Read the model definition and answer for the solid it produces. Units are mm, in the model's axes. A direction names the side the tool comes from. Coordinates: 2 decimals unless noted, no trailing zeros. Write each loop counter-clockwise with the first axis right and the second up, starting at its lowest first coordinate (ties: lowest second). Pieces come first, ordered by that corner, then holes.
Item 1: Straight lines are drawn through the part: probe 1 along Z at (x, y) = (163, 14.5); probe 2 along X at (y, z) = (22, 67); probe 3 along X at (y, z) = (21, 66.5). For each, find the intervals that lie inside material, in ascending order.
Item 2: Section B-B (z = 62.5) is taken. Give the vertices of the cut face in (x, y).
Item 3: Determine the mould class of faces 4 (the face through (151.284, 25, 35)), 5 (the face through (59.284, 24, 5)), 6 (the face through (168.441, 22.825, 5.07)) for opening direction X: released by +X, released by -X, zero draft, split by the parting line, or undercut.
Item 4: A tool of negligible diameter and unlimited length cuts with its end or side. For faces 1 (the face through (185.28, 24.75, 65.07)), 2 (the face through (169, 25, 10)), 3 (the face through (86.382, 24.269, 59.145)), from which of +Z, -Z, +X, -X, +Y, -Y can it reach the whole face along a straight path? Write none if from no direction.
Item 5: Section A-A (y = 35) is taken. Give the vertices of the cut face in (x, z).
Item 6: Each of these flat-tipped pins is pushed along its axis until it touches: P1, Ø11, axis at y = 22, z = 5.5, coming from the -X side; P2, Ø12, axis at y = 23, z = 38, coming from the +X side; P3, Ø3, axis at y = 26.5, z = 7.5, coming from the +X side. Where does it stop, or does it pass through?
Item 7: Section C-C (z = 27.5) is taken. Give the vertices of the cut face in (x, y).
from build123d import *

# Parameters (mm, degrees)
SKETCH_1_W             = 120
SKETCH_1_H             = 40
EXTRUDE_1_DEPTH        = 70
SKETCH_2_R             = 3
CUT_EXTRUDE_1_DEPTH    = 198.553816398
SKETCH_3_W             = 47.323469883
SKETCH_3_H             = 50
CUT_EXTRUDE_2_DEPTH    = 197.577989194
FILLET_1_R             = 3
SKETCH_4_W             = 12
SKETCH_4_H             = 40
EXTRUDE_2_DEPTH        = 10
SKETCH_5_W             = 12
SKETCH_5_H             = 40
EXTRUDE_3_DEPTH        = 10
SKETCH_6_R             = 3
EXTRUDE_4_DEPTH        = 10
SKETCH_7_R             = 4.5
CUT_EXTRUDE_3_DEPTH    = 10
CHAMFER_1_SIZE         = 2
HOLE_WIZARD_M8_1_D     = 9
HOLE_WIZARD_M8_1_DEPTH = 19.75
HOLE_WIZARD_M8_1_TIP   = 2.703872786


with BuildPart() as part:
    # 草图1 → 凸台-拉伸1 (new body)
    with BuildSketch(Plane.XY):
        with Locations((119.284427197, 24.548900527)):
            Rectangle(SKETCH_1_W, SKETCH_1_H)
    extrude(amount=EXTRUDE_1_DEPTH)

    # 草图2 → 切除-拉伸1 (cut, through all)
    with BuildSketch(Plane.XY.offset(70)):
        with Locations((74.284427197, 24.548900527)):
            Circle(SKETCH_2_R)
        with Locations((164.284427197, 24.548900527)):
            Circle(SKETCH_2_R)
    extrude(amount=-CUT_EXTRUDE_1_DEPTH, mode=Mode.SUBTRACT)

    # 草图3 → 切除-拉伸2 (cut, through all)
    with BuildSketch(Plane(origin=(0, 44.548900527, 0), x_dir=(1, 0, 0), z_dir=(0, 1, 0))):
        with Locations((174.946162139, -35)):
            Rectangle(SKETCH_3_W, SKETCH_3_H)
        with Locations((63.622692255, -35)):
            Rectangle(SKETCH_3_W, SKETCH_3_H)
    extrude(amount=-CUT_EXTRUDE_2_DEPTH, mode=Mode.SUBTRACT)

    # 圆角1
    fillet_1_edges = [part.edges().sort_by_distance(p)[0] for p in [
        (151.284427197, 24.548900527, 10),
        (151.284427197, 24.548900527, 60),
        (87.284427197, 24.548900527, 60),
        (87.284427197, 24.548900527, 10),
    ]]
    fillet(fillet_1_edges, radius=FILLET_1_R)

    # 草图4 → 凸台-拉伸2 (add)
    with BuildSketch(Plane(origin=(0, 0, 60), x_dir=(-1, 0, 0), z_dir=(0, 0, -1))):
        with Locations((-185.284427197, 24.548900527)):
            Rectangle(SKETCH_4_W, SKETCH_4_H)
    extrude(amount=-EXTRUDE_2_DEPTH)

    # 草图5 → 凸台-拉伸3 (add)
    with BuildSketch(Plane.XY.offset(70)):
        with Locations((53.284427197, 24.548900527)):
            Rectangle(SKETCH_5_W, SKETCH_5_H)
    extrude(amount=-EXTRUDE_3_DEPTH)

    # 草图6 → 凸台-拉伸4 (add)
    with BuildSketch(Plane.XY.offset(70)):
        with Locations((74.284427197, 24.548900527)):
            Circle(SKETCH_6_R)
        with Locations((164.284427197, 24.548900527)):
            Circle(SKETCH_6_R)
    extrude(amount=-EXTRUDE_4_DEPTH)

    # 草图7 → 切除-拉伸3 (cut)
    with BuildSketch(Plane.XY.offset(70)):
        with Locations((57.784427197, 24.548900527)):
            Circle(SKETCH_7_R)
    cut_extrude_3 = extrude(amount=-CUT_EXTRUDE_3_DEPTH, mode=Mode.SUBTRACT)

    # 镜向2: 切除-拉伸3 across plane
    add(cut_extrude_3.mirror(Plane(origin=(119.284427197, 0, 0), x_dir=(0, 0, 1), z_dir=(1, 0, 0))), mode=Mode.SUBTRACT)

    # 倒角1
    chamfer_1_edges = [part.edges().sort_by_distance(p)[0] for p in [
        (47.284427197, 4.548900527, 65),
        (47.284427197, 44.548900527, 65),
        (179.284427197, 4.548900527, 5),
        (179.284427197, 44.548900527, 5),
        (59.284427197, 4.548900527, 5),
        (59.284427197, 44.548900527, 5),
        (191.284427197, 4.548900527, 65),
        (191.284427197, 44.548900527, 65),
    ]]
    chamfer(chamfer_1_edges, length=CHAMFER_1_SIZE)

    # Hole Wizard M8 _1
    with Locations(Plane(origin=(74.284427197, 24.548900527, 0), x_dir=(-1, 0, 0), z_dir=(0, 0, -1))):
        with Locations((0, 0), (-90, 0)):
            Hole(HOLE_WIZARD_M8_1_D / 2, depth=HOLE_WIZARD_M8_1_DEPTH)
            with Locations((0, 0, -(HOLE_WIZARD_M8_1_DEPTH + HOLE_WIZARD_M8_1_TIP / 2))):  # 118° drill point
                Cone(0, HOLE_WIZARD_M8_1_D / 2, HOLE_WIZARD_M8_1_TIP, mode=Mode.SUBTRACT)


solid = part.part
Established:
1. probe 1: z = 0 to 10, 60 to 70
1. probe 2: x = 47.28 to 54.08, 61.49 to 177.08, 184.49 to 191.28
1. probe 3: x = 47.28 to 55.02, 60.55 to 178.02, 183.55 to 191.28
2. outline: (47.28, 6.55) - (49.28, 4.55) - (189.28, 4.55) - (191.28, 6.55) - (191.28, 42.55) - (189.28, 44.55) - (49.28, 44.55) - (47.28, 42.55) - close; hole circle Ø9 at (57.78, 24.55); hole circle Ø9 at (180.78, 24.55)
3. face 4: released by +X
3. face 5: released by -X
3. face 6: undercut
4. face 1: +Z
4. face 2: +X, +Y, -Y
4. face 3: -X, +Y, -Y
5. outline: (47.28, 60) - (84.28, 60) arc R3 cw to (87.28, 57) - (87.28, 13) arc R3 cw to (84.28, 10) - (59.28, 10) - (59.28, 0) - (179.28, 0) - (179.28, 10) - (154.28, 10) arc R3 cw to (151.28, 13) - (151.28, 57) arc R3 cw to (154.28, 60) - (191.28, 60) - (191.28, 70) - (47.28, 70) - close
6. P1: stops at x = 59.28
6. P2: stops at x = 151.28
6. P3: stops at x = 179.28
7. outline: (87.28, 4.55) - (151.28, 4.55) - (151.28, 44.55) - (87.28, 44.55) - close
